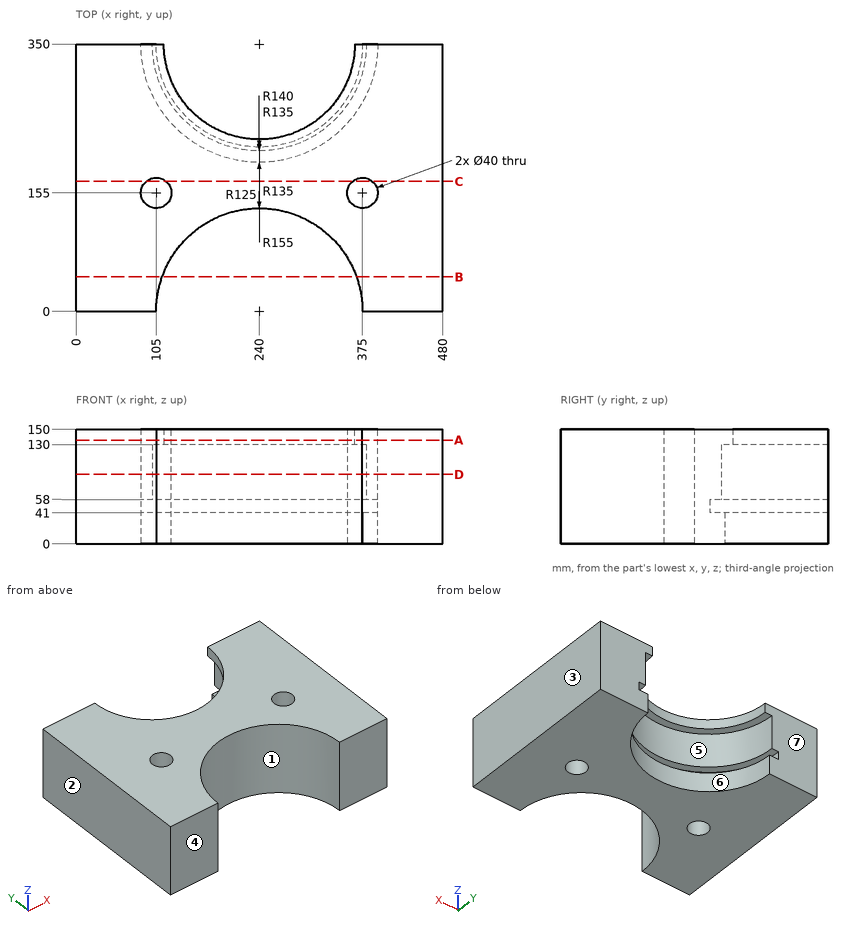
Answer from the drawing. Dimensions are ordinates in mm from the lowest x, y and z of the part. A direction names the side the tool comes from. Round coordinates to 2 decimals unless told otherwise and drop trailing zeros. Write each loop counter-clockwise with the first axis right and the second up, starting at its lowest first coordinate (ties: lowest second). Pieces come first, ordered by that corner, then holes. Notation, with made-up numbers: (57, -27) - (105, -27) arc R25 ccw to (105, 0) - close; hole circle Ø5 at (81.5, 38.5). An arc over 180 degrees is marked (long way). One line per item, written item: value.
Q1. This flat-tipped pin is pushed along its axis until it touches: P1, Ø4, axis at y = 193.5, z = 58, coming from the -X side. Where does it stop, or does it pass through?
The answers:
P1: stops at x = 0
Q2. Straight lines are drawn through the part: line 1 (X direction, y = 136.5, z = 84); line 2 (X direction, y = 158.5, z = 60.5); line 3 (Z direction, x = 126.5, y = 265). For each, find the intervals that lie inside material, in ascending order. Write a range as from..to.
The answers:
line 1: x = 0..97.4, 112.6..367.4, 382.6..480
line 2: x = 0..85.31, 124.69..355.31, 394.69..480
line 3: z = 0..41, 58..150
Q3. Find section B-B (y = 45). Determine the outline of the cut face in (x, z), and give its area (3 significant figures).
The answers:
outline: (0, 0) - (112.72, 0) - (112.72, 150) - (0, 150) - close; (367.28, 0) - (480, 0) - (480, 150) - (367.28, 150) - close
area: 33,800 mm2
Q4. Which of the six approach directions +Z, -Z, +X, -X, +Y, -Y give full straight-line access (tool end or side, diameter ignored) to the marked faces 5, 6 and 7?
The answers:
face 5: +Y
face 6: -Z, +Y
face 7: +Z, -Z, +X, -X, +Y
Q5. Find section C-C (y = 170). Determine the outline of the cut face in (x, z).
The answers:
outline: (0, 0) - (91.77, 0) - (91.77, 150) - (0, 150) - close; (118.23, 0) - (361.77, 0) - (361.77, 150) - (118.23, 150) - close; (388.23, 0) - (480, 0) - (480, 150) - (388.23, 150) - close
Q6. For a pull along X with two mould halves and no side action, classify the marked faces 1, 2, 3 and 4 as pulls with the +X half, pulls with the -X half, needs draft (parallel to the pull), parting line crosses it, or undercut.
The answers:
face 1: undercut
face 2: pulls with the -X half
face 3: pulls with the +X half
face 4: needs draft
Q7. Find section A-A (z = 136). Determine the outline of the cut face in (x, y), and give its area (3 significant figures).
The answers:
outline: (0, 0) - (105, 0) arc R135 cw to (375, 0) - (480, 0) - (480, 350) - (365, 350) arc R125 cw to (115, 350) - (0, 350) - close; hole circle Ø40 at (105, 155); hole circle Ø40 at (375, 155)
area: 112,000 mm2
Q8. Find section D-D (z = 91). Determine the outline of the cut face in (x, y), and give its area (3 significant figures).
The answers:
outline: (0, 0) - (105, 0) arc R135 cw to (375, 0) - (480, 0) - (480, 350) - (380, 350) arc R140 cw to (100, 350) - (0, 350) - close; hole circle Ø40 at (105, 155); hole circle Ø40 at (375, 155)
area: 106,000 mm2
